```python
from build123d import *

# Parameters (mm, degrees)
SKETCH_1_R          = 1.6
EXTRUDE_1_DEPTH     = 2
SKETCH_2_W          = 200
SKETCH_2_H          = 2
EXTRUDE_2_DEPTH     = 48
SKETCH_3_R          = 3.2
SKETCH_3_R_2        = 4.2
CUT_EXTRUDE_1_DEPTH = 48


with BuildPart() as part:
    # 草图1 → 凸台-拉伸1 (new body)
    with BuildSketch(Plane.XY):
        with BuildLine():
            Line((1437.273715593, 307.480108419), (1237.273715593, 307.480108419))
            Line((1237.273715593, 307.480108419), (1237.273715593, 361.14640389))
            ThreePointArc((1237.273715593, 361.14640389), (1337.273715593, 391.480108419), (1437.273715593, 361.14640389))
            Line((1437.273715593, 361.14640389), (1437.273715593, 307.480108419))
        make_face()
        with Locations((1337.273715593, 387.480108419)):
            Circle(SKETCH_1_R, mode=Mode.SUBTRACT)
        with Locations((1337.273715593, 380.480108419)):
            Circle(SKETCH_1_R, mode=Mode.SUBTRACT)
        with Locations((1321.934304869, 386.810375283)):
            Circle(SKETCH_1_R, mode=Mode.SUBTRACT)
        with Locations((1322.544395068, 379.837012397)):
            Circle(SKETCH_1_R, mode=Mode.SUBTRACT)
        with Locations((1306.711636323, 384.806272949)):
            Circle(SKETCH_1_R, mode=Mode.SUBTRACT)
        with Locations((1307.927173567, 377.912618678)):
            Circle(SKETCH_1_R, mode=Mode.SUBTRACT)
        with Locations((1291.721563655, 381.483053846)):
            Circle(SKETCH_1_R, mode=Mode.SUBTRACT)
        with Locations((1293.53329697, 374.721573062)):
            Circle(SKETCH_1_R, mode=Mode.SUBTRACT)
        with Locations((1277.078170367, 376.866009678)):
            Circle(SKETCH_1_R, mode=Mode.SUBTRACT)
        with Locations((1279.472311371, 370.288161332)):
            Circle(SKETCH_1_R, mode=Mode.SUBTRACT)
        with Locations((1262.892901526, 370.990278938)):
            Circle(SKETCH_1_R, mode=Mode.SUBTRACT)
        with Locations((1265.851229359, 364.646124428)):
            Circle(SKETCH_1_R, mode=Mode.SUBTRACT)
        with Locations((1249.273715593, 363.900579485)):
            Circle(SKETCH_1_R, mode=Mode.SUBTRACT)
        with Locations((1252.773715593, 357.838401659)):
            Circle(SKETCH_1_R, mode=Mode.SUBTRACT)
        with Locations((1425.273715593, 363.900579485)):
            Circle(SKETCH_1_R, mode=Mode.SUBTRACT)
        with Locations((1421.773715593, 357.838401659)):
            Circle(SKETCH_1_R, mode=Mode.SUBTRACT)
        with Locations((1411.654529659, 370.990278938)):
            Circle(SKETCH_1_R, mode=Mode.SUBTRACT)
        with Locations((1408.696201827, 364.646124428)):
            Circle(SKETCH_1_R, mode=Mode.SUBTRACT)
        with Locations((1397.469260818, 376.866009678)):
            Circle(SKETCH_1_R, mode=Mode.SUBTRACT)
        with Locations((1395.075119815, 370.288161332)):
            Circle(SKETCH_1_R, mode=Mode.SUBTRACT)
        with Locations((1382.825867531, 381.483053846)):
            Circle(SKETCH_1_R, mode=Mode.SUBTRACT)
        with Locations((1381.014134215, 374.721573062)):
            Circle(SKETCH_1_R, mode=Mode.SUBTRACT)
        with Locations((1367.835794862, 384.806272949)):
            Circle(SKETCH_1_R, mode=Mode.SUBTRACT)
        with Locations((1366.620257618, 377.912618678)):
            Circle(SKETCH_1_R, mode=Mode.SUBTRACT)
        with Locations((1352.613126316, 386.810375283)):
            Circle(SKETCH_1_R, mode=Mode.SUBTRACT)
        with Locations((1352.003036117, 379.837012397)):
            Circle(SKETCH_1_R, mode=Mode.SUBTRACT)
    extrude(amount=EXTRUDE_1_DEPTH)

    # 草图2 → 凸台-拉伸2 (add)
    with BuildSketch(Plane.XY.offset(2)):
        with Locations((1337.273715593, 308.480108419)):
            Rectangle(SKETCH_2_W, SKETCH_2_H)
    extrude(amount=EXTRUDE_2_DEPTH)

    # 草图3 → 切除-拉伸1 (cut)
    with BuildSketch(Plane(origin=(0, 309.480108419, 0), x_dir=(1, 0, 0), z_dir=(0, 1, 0))):
        with Locations(Location((1287.273715593, -30, 0), (0, 0, 270))):
            Circle(SKETCH_3_R)
        with Locations(Location((1387.273715593, -30, 0), (0, 0, 270))):
            Circle(SKETCH_3_R)
        with Locations(Location((1257.273715593, -15, 0), (0, 0, 270))):
            Circle(SKETCH_3_R_2)
        with Locations(Location((1417.273715593, -15, 0), (0, 0, 270))):
            Circle(SKETCH_3_R_2)
        with Locations(Location((1257.273715593, -30, 0), (0, 0, 270))):
            Circle(SKETCH_3_R_2)
        with Locations(Location((1287.273715593, -15, 0), (0, 0, 270))):
            Circle(SKETCH_3_R)
        with Locations(Location((1387.273715593, -15, 0), (0, 0, 270))):
            Circle(SKETCH_3_R)
        with Locations(Location((1417.273715593, -30, 0), (0, 0, 270))):
            Circle(SKETCH_3_R_2)
    extrude(amount=-CUT_EXTRUDE_1_DEPTH, mode=Mode.SUBTRACT)


solid = part.part
```
Geometry check sheet. Reference: the model listing, model coordinates, mm. A direction names the side the tool comes from. Coordinates: 2 decimals unless noted, no trailing zeros. Order: outer loops, then holes, each group sorted by start corner. A loop starts at its lowest first (then second) coordinate and runs counter-clockwise, first axis right, second up. Notation, with made-up numbers: (-32.5, 23.5) - (4.5, 23.5) arc R35 ccw to (4.5, 61.5) - close; hole circle Ø2 at (76, 51.5). An arc over 180 degrees is marked (long way). Answer as a JSON object with one key per item and string values. Group by question number.
Item 1: Tool access check on faces 1 (the face through (1336, 309.48, 26)), 2 (the face through (1413.55, 308.49, 31.94)). Record the directions out of +Z, -Z, +X, -X, +Y, -Y that give a thin tool (end or side, any length) a straight path to the whole face; none if there is none.
Item 2: Sectioned sample at C-C, the plane y = 324. Record the cut outline in (x, z).
Item 3: Sectioned sample at D-D, the plane z = 8.5. Record the cut outline in (x, y).
Item 4: Depth check by flat-ended pin: pin 1 Ø1 at (x, z) = (1272, 10.5) entering from +Y; pin 2 Ø4 at (x, y) = (1306.71, 384.81) entering from +Z. Enter the tip coordinate at first touch or a pass-through.
Item 5: Sectioned sample at A-A, the plane z = 30. Record the cut outline in (x, y), and give its area (3 significant figures).
Item 6: Scan lines: probe 1 along Z at (x, y) = (1315.5, 320); probe 2 along Y at (x, z) = (1382.5, 46). Record each from-to range of solid material in increasing order.
Item 7: Sectioned sample at B-B, the plane x = 1357. Record the cut outline in (y, z).
Item 8: Draft check along X on faces 3 (the face through (1437.274, 322, 1)), 4 (the face through (1237.274, 322, 1)), 5 (the face through (1413.55, 308.49, 16.94)), 6 (the face through (1339, 342, 2)). Enter one of: +X half, -X half, draft (parallel to the pull), parting line (faces both ways), or undercut.
Resolved:
{
 "1": {"face 1": "+Z, +X, -X, +Y", "face 2": "+Y, -Y"},
 "2": {"outline": "(1237.27, 0) - (1437.27, 0) - (1437.27, 2) - (1237.27, 2) - close"},
 "3": {"outline": "(1237.27, 307.48) - (1437.27, 307.48) - (1437.27, 309.48) - (1237.27, 309.48) - close"},
 "4": {"pin 1": "y = 309.48", "pin 2": "z = 2"},
 "5": {"outline": "(1237.27, 307.48) - (1253.07, 307.48) - (1253.07, 309.48) - (1237.27, 309.48) - close; (1261.47, 307.48) - (1284.07, 307.48) - (1284.07, 309.48) - (1261.47, 309.48) - close; (1290.47, 307.48) - (1384.07, 307.48) - (1384.07, 309.48) - (1290.47, 309.48) - close; (1390.47, 307.48) - (1413.07, 307.48) - (1413.07, 309.48) - (1390.47, 309.48) - close; (1421.47, 307.48) - (1437.27, 307.48) - (1437.27, 309.48) - (1421.47, 309.48) - close", "area": "341 mm^2"},
 "6": {"probe 1": "0 to 2", "probe 2": "307.48 to 309.48"},
 "7": {"outline": "(307.48, 0) - (390.4, 0) - (390.4, 2) - (309.48, 2) - (309.48, 50) - (307.48, 50) - close"},
 "8": {"face 3": "+X half", "face 4": "-X half", "face 5": "undercut", "face 6": "draft"}
}
